```python
from build123d import *
from build123d.topology import SkipClean

# Parameters (mm, degrees)
SKETCH1_R              = 15
BOSS_EXTRUDE1_DEPTH    = 140
SKETCH2_R              = 12
BOSS_EXTRUDE2_DEPTH    = 45
BOSS_EXTRUDE3_START    = 3
BOSS_EXTRUDE3_DEPTH    = 3
M10_TAPPED_HOLE1_D     = 8.5
M10_TAPPED_HOLE1_DEPTH = 24.5
M10_TAPPED_HOLE1_TIP   = 2.553657631
CHAMFER1_SIZE          = 1.5


with BuildPart() as part:
    # Sketch1 → Boss-Extrude1 (new body)
    with BuildSketch(Plane.XY):
        Circle(SKETCH1_R)
    extrude(amount=BOSS_EXTRUDE1_DEPTH)

    # Sketch2 → Boss-Extrude2 (add)
    with BuildSketch(Plane.XY.offset(140)):
        with Locations(Location((0, 0, 0), (0, 0, 180))):
            Circle(SKETCH2_R)
    extrude(amount=BOSS_EXTRUDE2_DEPTH)

    # Sketch3 → Boss-Extrude3 (add)
    with SkipClean():  # the faces are left unmerged after this step: merging them gives an invalid solid
        with BuildSketch(Plane(origin=(0, 0, 0), x_dir=(-1, 0, 0), z_dir=(0, 0, -1)).offset(BOSS_EXTRUDE3_START)):
            with BuildLine():
                Line((-6, 13.747727085), (-6, -13.747727085))
                ThreePointArc((-6, -13.747727085), (0, -15), (6, -13.747727085))
                Line((6, -13.747727085), (6, 13.747727085))
                ThreePointArc((6, 13.747727085), (0, 15), (-6, 13.747727085))
            make_face()
        extrude(amount=-BOSS_EXTRUDE3_DEPTH)

    # M10 Tapped Hole1
    with Locations(Plane(origin=(0, 0, -3), x_dir=(-1, 0, 0), z_dir=(0, 0, -1))):
        with Locations((0, 0)):
            Hole(M10_TAPPED_HOLE1_D / 2, depth=M10_TAPPED_HOLE1_DEPTH)
            with Locations((0, 0, -(M10_TAPPED_HOLE1_DEPTH + M10_TAPPED_HOLE1_TIP / 2))):  # 118° drill point
                Cone(0, M10_TAPPED_HOLE1_D / 2, M10_TAPPED_HOLE1_TIP, mode=Mode.SUBTRACT)

    # Chamfer1
    chamfer1_edges = [part.edges().sort_by_distance(p)[0] for p in [
        (12, 0, 185),
    ]]
    chamfer(chamfer1_edges, length=CHAMFER1_SIZE)


solid = part.part
```
Verification items for the finished model (mm, model axes). A direction names the side the tool comes from. Round coordinates to 2 decimals unless told otherwise and drop trailing zeros. Write each loop counter-clockwise with the first axis right and the second up, starting at its lowest first coordinate (ties: lowest second). Pieces come first, ordered by that corner, then holes. Notation, with made-up numbers: (88.25, 36) - (113.25, 36) arc R37 cw to (113.25, 74) - close; hole circle Ø10 at (63, 20.5). An arc over 180 degrees is marked (long way). Answer as a JSON object with one key per item and string values. Group by question number.
Q1. Section check B-B, the plane z = 144. Enter the section's corners in (x, y).
Q2. Section check A-A, the plane z = 13.5. Enter the section's corners in (x, y).
Q3. Tool access check on faces 4 (the flat face through (6, 0, -2)), 5 (the flat face through (-7, 10, 140)), 6 (the flat face through (-10, 0, 0)). Record the directions out of +Z, -Z, +X, -X, +Y, -Y that give a thin tool (end or side, any length) a straight path to the whole face; none if there is none.
Q4. Section check C-C, the plane z = 99. Enter the section's corners in (x, y).
Q5. Thickness scan on line 1 (X direction, y = 0, z = 12.25); line 2 (Z direction, x = 0, y = 13.75). Record the ranges inside material, lowest first.
Q6. Go/stop test with flat-tipped pins: pin 1 Ø1 at (y, z) = (10.5, 66) entering from +X; pin 2 Ø1.5 at (y, z) = (5, 129.5) entering from -X; pin 3 Ø5 at (x, z) = (-11, 102) entering from -Y. Record where each tip stops, or that it passes through.
Q7. Mould release check, pull along Y, two halves, no side actions. Record for faces 1 (the cylindrical face through (2.285, 3.584, 9.422)), 2 (the flat face through (-6, 0, -2)), 3 (the cylindrical face through (-11.446, -3.604, 161.446)): released by +Y, released by -Y, zero draft, split by the parting line, or undercut.
Found:
{
 "1": {"outline": "circle Ø24 at (0, 0)"},
 "2": {"outline": "circle Ø30 at (0, 0); hole circle Ø8.5 at (0, 0)"},
 "3": {"face 4": "-Z, +X, +Y, -Y", "face 5": "+Z", "face 6": "-Z, -X, +Y, -Y"},
 "4": {"outline": "circle Ø30 at (0, 0)"},
 "5": {"line 1": "x = -15 to -4.25, 4.25 to 15", "line 2": "z = -3 to 140"},
 "6": {"pin 1": "stops at x = 11.18", "pin 2": "stops at x = -14.39", "pin 3": "stops at y = -12.36"},
 "7": {"face 1": "undercut", "face 2": "zero draft", "face 3": "split by the parting line"}
}
